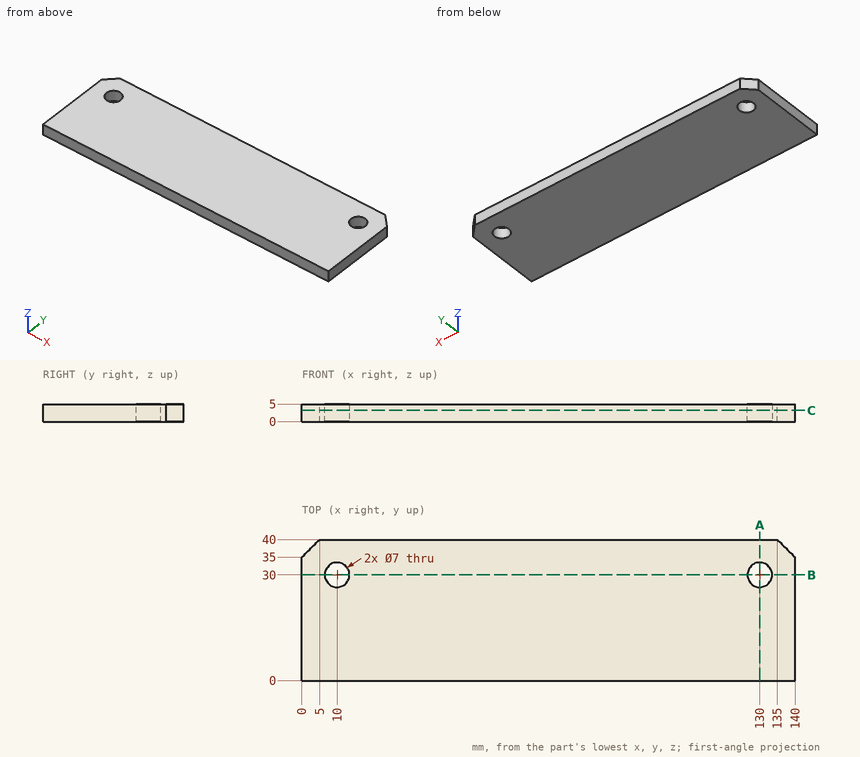
Drawing for the job (mm, zero at the part's lowest x, y, z). Give positions to 0.01 mm unless a question says otherwise; leave off trailing zeros. Loops run counter-clockwise (first coordinate to the right, second up) from the corner with the lowest first, then second, coordinate; pieces in that order, holes last.
1) Drop a flat-ended pin along its axis: P1, Ø10, axis at x = 63, y = 14, coming from the -Z side. Give the stop position or say it passes through.
Values follow:
P1: stops at z = 0
2) Probe line 1 along Y through (x, z) = (130, 2.05). List the from-to ranges inside material, lowest first.
Values follow:
line 1: y = 0 to 26.5, 33.5 to 40
3) Band-saw the part on C-C on z = 3.2. List the corners of the cut face in (x, y), then the cut area to 3 significant figures.
Values follow:
outline: (0, 0) - (140, 0) - (140, 35) - (135, 40) - (5, 40) - (0, 35) - close; hole circle Ø7 at (10, 30); hole circle Ø7 at (130, 30)
area: 5,500 mm2
4) Band-saw the part on A-A on x = 130. List the corners of the cut face in (y, z).
Values follow:
outline: (0, 0) - (26.5, 0) - (26.5, 5) - (0, 5) - close; (33.5, 0) - (40, 0) - (40, 5) - (33.5, 5) - close
5) Band-saw the part on B-B on y = 30. List the corners of the cut face in (x, z).
Values follow:
outline: (0, 0) - (6.5, 0) - (6.5, 5) - (0, 5) - close; (13.5, 0) - (126.5, 0) - (126.5, 5) - (13.5, 5) - close; (133.5, 0) - (140, 0) - (140, 5) - (133.5, 5) - close
